Part model, mm, in its own coordinate system. A direction names the side the tool comes from. Coordinates: 2 decimals unless noted, no trailing zeros. Loops run counter-clockwise (first coordinate to the right, second up) from the corner with the lowest first, then second, coordinate; pieces in that order, holes last. Notation, with made-up numbers: (71.25, 81.5) -> (116.25, 81.5) arc R10 cw to (116.25, 97.5) -> close; hole circle Ø3 at (47, -2.5). An arc over 180 degrees is marked (long way). Use one line per item in the form item = value. Start each with the question number.
(1) Band-saw the part on D-D on x = 717. Give the cut face in (y, z), then the cut area to 3 significant figures.
(2) Mould opens along Y. For faces 1 (the flat face through (423, -40, 0)), 2 (the flat face through (382, 0, -17)), 3 (the flat face through (382, 0, 17)), 4 (the flat face through (382, 0, -20)) say: +Y half, -Y half, draft (parallel to the pull), parting line (faces both ways), or undercut.
(3) Pin check, flat tip, straight feed: P1, Ø1.5, axis at x = 275, z = 15, coming from the -Y side. Stop position of the tip, or through.
(4) Band-saw the part on A-A on z = 7. Give the cut face in (x, y), then the cut area to 3 significant figures.
(5) Band-saw the part on C-C on x = 549.5. Give the cut face in (y, z), then the cut area to 3 significant figures.
(6) 3-axis set-ups, long thin cutter, end or side, ignore diameter. For faces 5 (the flat face through (420, -37, 0)), 6 (the flat face through (343, 40, 0)): which of +Z, -Z, +X, -X, +Y, -Y reach the whole face in a straight line?
(7) Band-saw the part on B-B on y = 13. Give the cut face in (x, z), then the cut area to 3 significant figures.
(8) Drill centre lines: L1, parallel to Z at x = 327.5, y = -17; L2, parallel to Y at x = 305.5, z = 8; L3, parallel to Y at x = 735.5, z = -0.5. Where is each one in solid material? Low to high. Write a range as [from, to].
```python
from build123d import *

# Parameters (mm, degrees)
COLD_FORMED_RECT_HOLLOW_SECTION_GB_T_672_DEPTH = 775
CUT_EXTRUDE1_DEPTH                             = 778.061773606


with BuildPart() as part:
    # Sketch1 → Cold-Formed Rect Hollow Section GB/T 6728-2002 80 X 40 X 3(1) (new body)
    with BuildSketch(Plane(origin=(0, 0, 0), x_dir=(0, 0, -1), z_dir=(1, 0, 0))):
        with BuildLine():
            Line((-14, -40), (14, -40))
            ThreePointArc((14, -40), (18.242640687, -38.242640687), (20, -34))
            Line((20, -34), (20, 34))
            ThreePointArc((20, 34), (18.242640687, 38.242640687), (14, 40))
            Line((14, 40), (-14, 40))
            ThreePointArc((-14, 40), (-18.242640687, 38.242640687), (-20, 34))
            Line((-20, 34), (-20, -34))
            ThreePointArc((-20, -34), (-18.242640687, -38.242640687), (-14, -40))
        make_face()
        with BuildLine():
            Line((-14, -37), (14, -37))
            ThreePointArc((14, -37), (16.121320344, -36.121320344), (17, -34))
            Line((17, -34), (17, 34))
            ThreePointArc((17, 34), (16.121320344, 36.121320344), (14, 37))
            Line((14, 37), (-14, 37))
            ThreePointArc((-14, 37), (-16.121320344, 36.121320344), (-17, 34))
            Line((-17, 34), (-17, -34))
            ThreePointArc((-17, -34), (-16.121320344, -36.121320344), (-14, -37))
        make_face(mode=Mode.SUBTRACT)
    extrude(amount=COLD_FORMED_RECT_HOLLOW_SECTION_GB_T_672_DEPTH)

    # Sketch2 → Cut-Extrude1 (cut, through all)
    with BuildSketch(Plane.XY.offset(20)):
        Polygon((0, 40), (80, -40), (0, -40), (0, -34), (0, 34), align=None)
        Polygon((775, 40), (695, 40), (775, -40), align=None)
    extrude(amount=-CUT_EXTRUDE1_DEPTH, mode=Mode.SUBTRACT)


solid = part.part
```
A:
q1.outline = (-40, -14) arc R6 ccw to (-34, -20) -> (18, -20) -> (18, -17) -> (-34, -17) arc R3 cw to (-37, -14) -> (-37, 14) arc R3 cw to (-34, 17) -> (18, 17) -> (18, 20) -> (-34, 20) arc R6 ccw to (-40, 14) -> close
q1.area = 438 mm²
q2.face_1 = -Y half
q2.face_2 = undercut
q2.face_3 = undercut
q2.face_4 = draft
q3.P1 = -39.99
q4.outline = (0, 40) -> (3, 37) -> (698, 37) -> (695, 40) -> close; (77, -37) -> (80, -40) -> (775, -40) -> (772, -37) -> close
q4.area = 4,170 mm²
q5.outline = (-40, -14) arc R6 ccw to (-34, -20) -> (34, -20) arc R6 ccw to (40, -14) -> (40, 14) arc R6 ccw to (34, 20) -> (-34, 20) arc R6 ccw to (-40, 14) -> close; hole (-37, -14) arc R3 ccw to (-34, -17) -> (34, -17) arc R3 ccw to (37, -14) -> (37, 14) arc R3 ccw to (34, 17) -> (-34, 17) arc R3 ccw to (-37, 14) -> close
q5.area = 661 mm²
q6.face_5 = +X, -X
q6.face_6 = +Z, -Z, +X, -X, +Y
q7.outline = (27, -20) -> (722, -20) -> (722, -17) -> (27, -17) -> close; (27, 17) -> (722, 17) -> (722, 20) -> (27, 20) -> close
q7.area = 4,170 mm²
q8.L1 = [-20, -17], [17, 20]
q8.L2 = [-40, -37], [37, 40]
q8.L3 = [-40, -37]
